The drawing under review shows one solid part. Ordinate dimensions are in mm from its lowest x, y, z. A direction names the side the tool comes from. Round coordinates to 2 decimals unless told otherwise and drop trailing zeros. Write each loop counter-clockwise with the first axis right and the second up, starting at its lowest first coordinate (ties: lowest second). Pieces come first, ordered by that corner, then holes. Notation, with made-up numbers: M 25,-4 L 80,-4 A34 cw 80,26 Z; hole C -22.75,13 d10. An arc over 180 degrees is marked long. Write item = value, one per line. Start each with the question number.
Item 1: Take a section at C-C, the plane x = 10.5. Give the boundary of the cut face in (y, z).
Item 2: To check wall thickness, follow line 1 along Y through (x, z) = (17.5, 32); line 2 along Z through (x, y) = (5.5, 62.5); line 3 along Z through (x, y) = (3.5, 133). State the ranges of each line that lie inside material, in increasing order.
Item 3: The part is to be moulded in two halves that separate along Z. For the marked faces 1, 2 and 3, say which applies: +Z half, -Z half, draft (parallel to the pull), parting line (faces both ways), or undercut.
Item 4: For pin 1 Ø9 at (y, z) = (137.5, 35.05) entering from +X; pin 2 Ø6 at (x, y) = (21.5, 68.5) entering from +Z; pin 3 Ø6 at (x, y) = (12.5, 140) entering from -Z; pin 4 Ø5 at (x, y) = (6.5, 46) entering from +Z, all flat-tipped, find the tip position at first contact; note any pin that passes through.
Item 5: Take a section at B-B, the plane z = 100. Give the boundary of the cut face in (x, y).
Item 6: Take a section at D-D, the plane x = 26. Give the boundary of the cut face in (y, z), plus the area to 3 significant figures.
Item 7: Tool access review of the marked faces 4 and 5: name each direction out of +Z, -Z, +X, -X, +Y, -Y from which nothing blocks a thin tool from reaching the whole face with its end or side.
Item 8: Take a section at A-A, the plane y = 100. Give the boundary of the cut face in (x, z).
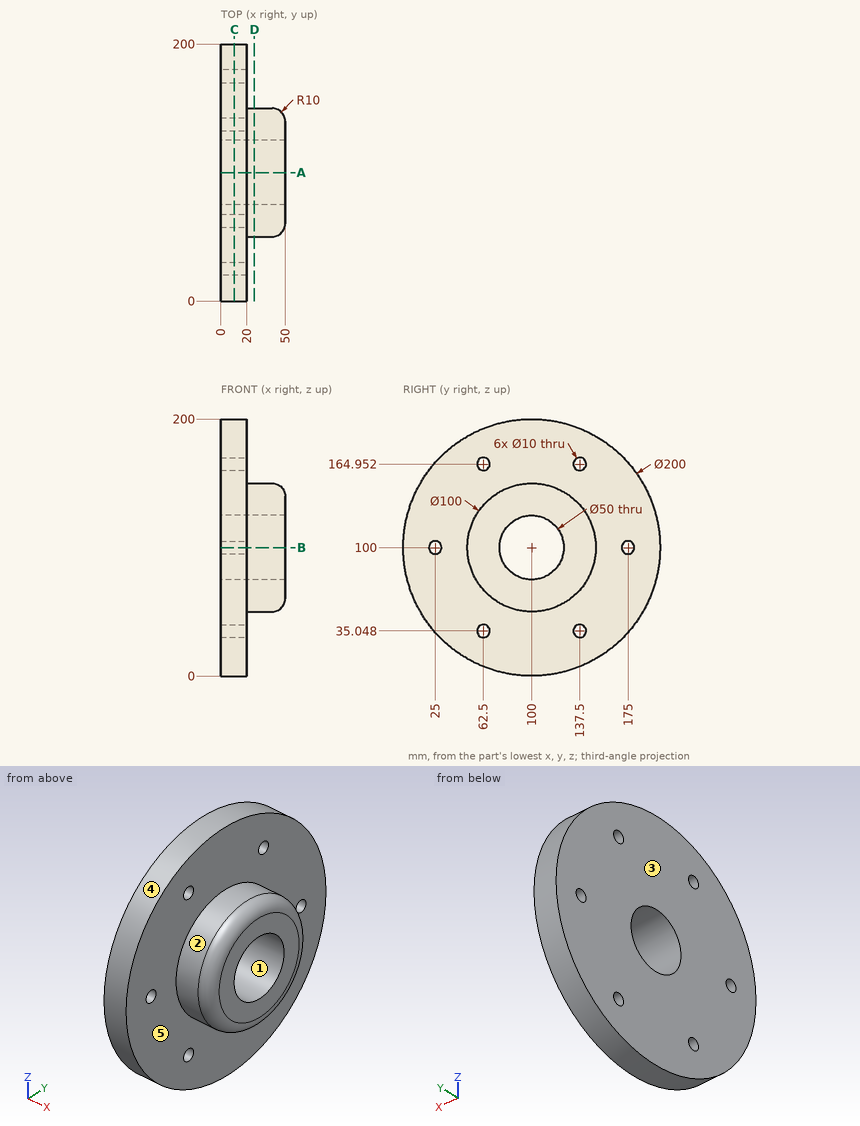
Response values:
q1.outline = C 100,100 d200; hole C 25,100 d10; hole C 62.5,35.05 d10; hole C 62.5,164.95 d10; hole C 100,100 d50; hole C 137.5,35.05 d10; hole C 137.5,164.95 d10; hole C 175,100 d10
q2.line_1 = 26.68 to 58.54, 66.46 to 133.54, 141.46 to 173.32
q2.line_2 = 7.3 to 30.05, 40.05 to 159.95, 169.95 to 192.7
q2.line_3 = 5.6 to 32.87, 37.23 to 162.77, 167.13 to 194.4
q3.face_1 = undercut
q3.face_2 = parting line
q3.face_3 = draft
q4.pin_1 = through
q4.pin_2 = 195.73
q4.pin_3 = 7.1
q4.pin_4 = 185.72
q5.outline = M 0,0 L 20,0 L 20,20 L 0,20 Z; M 0,30 L 20,30 L 20,50 L 40,50 A10 ccw 50,60 L 50,75 L 0,75 Z; M 0,125 L 50,125 L 50,140 A10 ccw 40,150 L 20,150 L 20,170 L 0,170 Z; M 0,180 L 20,180 L 20,200 L 0,200 Z
q6.outline = C 100,100 d100; hole C 100,100 d50
q6.area = 5,890 mm2
q7.face_4 = +X, -X
q7.face_5 = +X
q8.outline = M 0,0 L 20,0 L 20,50 L 40,50 A10 ccw 50,60 L 50,75 L 0,75 Z; M 0,125 L 50,125 L 50,140 A10 ccw 40,150 L 20,150 L 20,200 L 0,200 Z
